The listing builds one solid part. Answer for the finished solid, in the listing's coordinates (mm). A direction names the side the tool comes from. Coordinates: 2 decimals unless noted, no trailing zeros. Order: outer loops, then holes, each group sorted by start corner. A loop starts at its lowest first (then second) coordinate and runs counter-clockwise, first axis right, second up. Notation, with made-up numbers: (4.5, 38.5) -> (19.5, 38.5) arc R27 cw to (19.5, 68.5) -> close; hole circle Ø6 at (4, -10). An arc over 180 degrees is marked (long way). Return JSON: item names as keys, results as strings.
from build123d import *

# Parameters (mm, degrees)
EXTRUDE1_DEPTH = 664.7
SKETCH2_W      = 10
SKETCH2_H      = 50.8
SKETCH2_H_2    = 189.8
CHAMFER1_SIZE  = 1.5
CHAMFER2_SIZE  = 3


with BuildPart() as part:
    # Sketch1 → Extrude1 (new body)
    with BuildSketch(Plane.XY):
        Polygon((-22.627416998, 0), (0, 22.627416998), (22.627416998, 0), (0, -22.627416998), align=None)
    extrude(amount=EXTRUDE1_DEPTH)

    # Sketch2 → Cut-Revolve1 (revolve, cut)
    with BuildSketch(Plane(origin=(0, 0, 0), x_dir=(1, 0, 0), z_dir=(0, 1, 0)), mode=Mode.PRIVATE) as cut_revolve1_sk:
        with Locations((19.2875, -25.4)):
            Rectangle(SKETCH2_W, SKETCH2_H)
        with Locations((19.2875, -569.8)):
            Rectangle(SKETCH2_W, SKETCH2_H_2)
    revolve(cut_revolve1_sk.sketch.rotate(Axis((0, 0, 0), (0, 0, 1)), 180), axis=Axis((0, 0, 0), (0, 0, 1)), mode=Mode.SUBTRACT)

    # Chamfer1
    chamfer1_edges = [part.edges().sort_by_distance(p)[0] for p in [
        (14.2875, 0, 0),
    ]]
    chamfer(chamfer1_edges, length=CHAMFER1_SIZE)

    # Chamfer2
    chamfer2_edges = [part.edges().sort_by_distance(p)[0] for p in [
        (14.2875, 0, 664.7),
    ]]
    chamfer(chamfer2_edges, length=CHAMFER2_SIZE)


solid = part.part
1. For faces 1 (the face through (-11.47, 11.16, 259.88)), 2 (the face through (-5, -14, 474.9)), 3 (the face through (11.34, 8.69, 25.8)), determine the directions among +Z, -Z, +X, -X, +Y, -Y from which every point of the face is accessible in a straight line to the end or side of a thin tool.
Answer block:
{"face 1": "+Z, -Z, -X, +Y", "face 2": "+Z", "face 3": "-Z"}
2. Consider line 1 (Z direction, x = -15, y = -5); line 2 (Z direction, x = -11, y = -3); line 3 (Y direction, x = -13.5, z = 167). Determine where each line is inside the solid, lowest interval first. Write a range as from..to.
Answer block:
{"line 1": "z = 50.8..474.9", "line 2": "z = 0..664.59", "line 3": "y = -9.13..9.13"}
3. Each of these flat-tipped pins is pushed along its axis until it touches: pin 1 Ø5 at (y, z) = (-12.5, 174.5) entering from +X; pin 2 Ø1.5 at (x, z) = (-9.5, 70) entering from +Y; pin 3 Ø10 at (y, z) = (-9, 83) entering from +X; pin 4 Ø3 at (x, z) = (-16.5, 550.5) entering from +Y. Where does it stop, or does it pass through?
Answer block:
{"pin 1": "stops at x = 12.63", "pin 2": "stops at y = 13.88", "pin 3": "stops at x = 18.63", "pin 4": "passes through"}
4. The part is cut by section A-A on z = 423. Give the vertices of the cut face in (x, y), and give its area (3 significant figures).
Answer block:
{"outline": "(-22.63, 0) -> (0, -22.63) -> (22.63, 0) -> (0, 22.63) -> close", "area": "1,020 mm2"}
